from build123d import *

# Parameters (mm, degrees)
CIRPATTERN1_COUNT  = 4
CHAMFER1_SIZE      = 0.4
SKETCH8_R          = 6.5
CUT_EXTRUDE1_DEPTH = 10
SKETCH9_R          = 33
SKETCH9_R_2        = 32.25
CUT_EXTRUDE2_DEPTH = 10


with BuildPart() as part:
    # Sketch1 → Revolve1 (revolve)
    with BuildSketch(Plane.XY, mode=Mode.PRIVATE) as revolve1_sk:
        Polygon((0, 16), (1.695369244, 16), (1.695369244, 16.85), (2.995369244, 16.85), (2.995369244, 16), (13, 16), (13, 12.5), (15, 12.5), (15, 0), (18, 0), (18, 32.5), (14, 32.5), (14, 20), (0, 20), align=None)
    revolve(revolve1_sk.sketch.rotate(Axis((15, 0, 0), (1, 0, 0)), 90), axis=Axis((15, 0, 0), (1, 0, 0)))

    # Sketch2 → Cut-Revolve1 (revolve, cut)
    with BuildSketch(Plane(origin=(0, 0, 0), x_dir=(1, 0, 0), z_dir=(0, 1, 0)), mode=Mode.PRIVATE) as cut_revolve1_sk:
        Polygon((14, 26.5), (18, 26.5), (18, 31), (15.75, 28.75), (14, 28.75), align=None)
    cut_revolve1 = revolve(cut_revolve1_sk.sketch.rotate(Axis((14, 0, -26.5), (1, 0, 0)), 180), axis=Axis((14, 0, -26.5), (1, 0, 0)), mode=Mode.SUBTRACT)

    # CirPattern1: Cut-Revolve1 ×4 about axis
    cirpattern1_axis = Axis((0, 0, 0), (1, 0, 0))
    for i in range(1, CIRPATTERN1_COUNT):
        add(cut_revolve1.rotate(cirpattern1_axis, i * 360 / CIRPATTERN1_COUNT), mode=Mode.SUBTRACT)

    # Chamfer1
    chamfer1_edges = [part.edges().sort_by_distance(p)[0] for p in [
        (14, 0, -32.5),
        (18, 0, -32.5),
        (13, 0, -12.5),
        (0, 0, -16),
        (0, 0, -20),
    ]]
    chamfer(chamfer1_edges, length=CHAMFER1_SIZE)

    # Sketch8 → Cut-Extrude1 (cut)
    with BuildSketch(Plane.ZY.offset(-15)):
        Circle(SKETCH8_R)
    extrude(amount=-CUT_EXTRUDE1_DEPTH, mode=Mode.SUBTRACT)

    # Sketch9 → Cut-Extrude2 (cut)
    with BuildSketch(Plane(origin=(18, 0, 0), x_dir=(0, 0, -1), z_dir=(1, 0, 0))):
        Circle(SKETCH9_R)
        Circle(SKETCH9_R_2, mode=Mode.SUBTRACT)
    extrude(amount=-CUT_EXTRUDE2_DEPTH, mode=Mode.SUBTRACT)


solid = part.part
Geometry: final body of the model. Coordinates: model frame, mm. A direction names the side the tool comes from. Give positions to 0.01 mm unless a question says otherwise; leave off trailing zeros. Write each loop counter-clockwise with the first axis right and the second up, starting at its lowest first coordinate (ties: lowest second). Pieces come first, ordered by that corner, then holes. Notation, with made-up numbers: (71, 85) -> (97, 85) arc R27 cw to (97, 123) -> close; hole circle Ø7 at (-28, 57). An arc over 180 degrees is marked (long way). Answer as a JSON object with one key per item and string values.
1. Mould query, pull axis Y, two halves, no side actions, for faces 1 (the flat face through (1.695, 6, -15)), 2 (the cylindrical face through (16.03, 9.69, -30.76)), 3 (the flat face through (18, 7, 0)). Classes: pulls with the +Y half, pulls with the -Y half, needs draft (parallel to the pull), parting line crosses it, or undercut.
Ans:
{"face 1": "undercut", "face 2": "parting line crosses it", "face 3": "needs draft"}
2. Ray query, probe 1 along X at (y, z) = (-7, 7.5); probe 2 along Z at (x, y) = (15.5, 6); probe 3 along Y at (x, z) = (11.25, -12.5). Return the intervals inside material, ascending. Write a range as from..to.
Ans:
{"probe 1": "x = 15..18", "probe 2": "z = -31.69..-2.5, 2.5..31.69", "probe 3": "y = -15.61..-9.99, 9.99..15.61"}
3. Contact query for flat-ended pins moving along their axis: pin 1 (6 mm diameter, centred on y = 0, z = 26.5, fed in from +X); pin 2 (10 mm diameter, centred on x = 15.5, y = -9, fed in from -Z); pin 3 (1.5 mm diameter, centred on x = 7, z = -8.5, fed in from +Y). Output: stop coordinate, or through.
Ans:
{"pin 1": "stops at x = 16.5", "pin 2": "stops at z = -32", "pin 3": "stops at y = 18.44"}
4. Access query for faces 4 (the flat face through (2.995, 15, 6)), 5 (the cylindrical face through (8.07, 15.62, -3.47)), 6 (the conical face through (16, 29, 0)). Directions: +Z, -Z, +X, -X, +Y, -Y. A direction counts if a zero-diameter tool reaches every point of the face in a straight line with its end or side. Return the directions, or none.
Ans:
{"face 4": "none", "face 5": "-X", "face 6": "+X"}
5. Cut plane B-B on x = 8. Output: boundary loops of the cut face in (y, z).
Ans:
{"outline": "circle Ø40 at (0, 0); hole circle Ø32 at (0, 0)"}
6. Cut plane A-A on y = 0. Count the separate pieces of the cut face and the enclosed holes in it, and give its area (3 significant figures).
Ans:
{"separate pieces": "4", "enclosed holes": "0", "area": "264 mm^2"}
